Work out the finished part from the listing and answer in its coordinate system (mm). A direction names the side the tool comes from. Coordinates: 2 decimals unless noted, no trailing zeros. Order: outer loops, then holes, each group sorted by start corner. A loop starts at its lowest first (then second) coordinate and runs counter-clockwise, first axis right, second up. Notation, with made-up numbers: (-7, 84) -> (38, 84) arc R9 cw to (38, 97) -> close; hole circle Ø4 at (78, 66.5). An arc over 180 degrees is marked (long way). Use one line per item in the form item = value.
from build123d import *

# Parameters (mm, degrees)
KEYWAY_6X20_DEPTH_3_DEPTH = 3


with BuildPart() as part:
    # Shaft Profile Sketch → Stepped Shaft Body (revolve)
    with BuildSketch(Plane.XY, mode=Mode.PRIVATE) as stepped_shaft_body_sk:
        Polygon((0, 0), (130, 0), (130, -10), (30, -10), (30, -12.5), (20, -12.5), (20, -8.5), (15, -8.5), (15, -7), (7, -7), (7, -8.5), (0, -8.5), align=None)
    revolve(stepped_shaft_body_sk.sketch.rotate(Axis((0, 0, 0), (1, 0, 0)), 270), axis=Axis((0, 0, 0), (1, 0, 0)))

    # Keyway Sketch → Keyway 6x20 Depth 3 (cut)
    with BuildSketch(Plane.XY.offset(10)):
        Polygon((110, 0), (110, 3), (130, 3), (130, -3), (110, -3), align=None)
    extrude(amount=-KEYWAY_6X20_DEPTH_3_DEPTH, mode=Mode.SUBTRACT)


solid = part.part
(1) Each of these flat-tipped pins is pushed along its axis until it touches: P1, Ø1.5, axis at y = -1, z = 8, coming from the +X side; P2, Ø3, axis at x = 116.5, z = 8, coming from the +Y side; P3, Ø6, axis at x = 73, z = -3, coming from the +Y side. Where does it stop, or does it pass through?
Data:
P1 = 110
P2 = 7.6
P3 = 10
(2) Which of the six approach directions +Z, -Z, +X, -X, +Y, -Y give full straight-line access (tool end or side, diameter ignored) to faces 4 (the flat face through (15, -7, 2)), 5 (the cylindrical face through (79.3, 9.76, -2.17)), 6 (the flat face through (120, -3, 8))?
Data:
face_4 = none
face_5 = +X
face_6 = +Z, +X
(3) Section D-D on x = 61.5 is taken. Write down the section's boundary in (y, z).
Data:
outline = circle Ø20 at (0, 0)
(4) The mould has two halves that part along Y. Classify faces 1 (the flat face through (110, 0, 9)), 2 (the flat face through (20, 8.2, -3)), 3 (the cylindrical face through (3.451, -8.428, -1.107)): released by +Y, released by -Y, zero draft, split by the parting line, or undercut.
Data:
face_1 = undercut
face_2 = zero draft
face_3 = split by the parting line
(5) Straight lines are drawn through the part: line 1 along X through (y, z) = (-8, 7.25); line 2 along X through (y, z) = (-9.25, 1.75); line 3 along Y through (x, z) = (72, 0.25). For each, find the intervals that lie inside material, in ascending order.
Data:
line_1 = 20 to 30
line_2 = 20 to 130
line_3 = -10 to 10
(6) Section B-B on z = 0 is taken. Write down the section's boundary in (x, y).
Data:
outline = (0, -8.5) -> (7, -8.5) -> (7, -7) -> (15, -7) -> (15, -8.5) -> (20, -8.5) -> (20, -12.5) -> (30, -12.5) -> (30, -10) -> (130, -10) -> (130, 10) -> (30, 10) -> (30, 12.5) -> (20, 12.5) -> (20, 8.5) -> (15, 8.5) -> (15, 7) -> (7, 7) -> (7, 8.5) -> (0, 8.5) -> close
(7) Section C-C on x = 112 is taken. Write down the section's boundary in (y, z).
Data:
outline = (-3, 7) -> (-3, 9.54) arc R10 ccw (long way) to (3, 9.54) -> (3, 7) -> close
(8) Section A-A on y = 0 is taken. Write down the section's boundary in (x, z), plus the area to 3 significant figures.
Data:
outline = (0, -8.5) -> (7, -8.5) -> (7, -7) -> (15, -7) -> (15, -8.5) -> (20, -8.5) -> (20, -12.5) -> (30, -12.5) -> (30, -10) -> (130, -10) -> (130, 7) -> (110, 7) -> (110, 10) -> (30, 10) -> (30, 12.5) -> (20, 12.5) -> (20, 8.5) -> (15, 8.5) -> (15, 7) -> (7, 7) -> (7, 8.5) -> (0, 8.5) -> close
area = 2,510 mm²
